Read the model definition and answer for the solid it produces. Units are mm, in the model's axes. Coordinates: 2 decimals unless noted, no trailing zeros. Order: outer loops, then holes, each group sorted by start corner. A loop starts at its lowest first (then second) coordinate and runs counter-clockwise, first axis right, second up. Notation, with made-up numbers: (28.25, 54.5) -> (33.25, 54.5) arc R15 cw to (33.25, 74.5) -> close; hole circle Ø3 at (47.25, 21). An arc over 180 degrees is marked (long way). Answer in a Markdown table with one row per item.
from build123d import *

# Parameters (mm, degrees)
SKETCH1_W           = 300
SKETCH1_H           = 80
BOSS_EXTRUDE1_DEPTH = 8
SKETCH2_R           = 4
CUT_EXTRUDE1_DEPTH  = 8
CHAMFER1_SIZE       = 5


with BuildPart() as part:
    # Sketch1 → Boss-Extrude1 (new body)
    with BuildSketch(Plane.XY):
        Rectangle(SKETCH1_W, SKETCH1_H)
    extrude(amount=BOSS_EXTRUDE1_DEPTH)

    # Sketch2 → Cut-Extrude1 (cut)
    with BuildSketch(Plane.XY.offset(8)):
        with Locations((-137.5, 25)):
            Circle(SKETCH2_R)
        with Locations((-137.5, -25)):
            Circle(SKETCH2_R)
        with Locations((137.5, 25)):
            Circle(SKETCH2_R)
        with Locations((137.5, -25)):
            Circle(SKETCH2_R)
    extrude(amount=-CUT_EXTRUDE1_DEPTH, mode=Mode.SUBTRACT)

    # Chamfer1
    chamfer1_edges = [part.edges().sort_by_distance(p)[0] for p in [
        (-150, -40, 4),
        (-150, 40, 4),
        (150, 40, 4),
        (150, -40, 4),
    ]]
    chamfer(chamfer1_edges, length=CHAMFER1_SIZE)


solid = part.part
Q1. For a pull along X with two mould halves and no side action, classify faces 1 (the face through (-147, 38, 4)), 2 (the face through (-133.685, -23.799, 4.056)), 3 (the face through (-2, -40, 4)) as pulls with the +X half, pulls with the -X half, needs draft (parallel to the pull), parting line crosses it, or undercut.
Outcome:
| item | result |
|---|---|
| face 1 | pulls with the -X half |
| face 2 | undercut |
| face 3 | needs draft |
Q2. The part is cut by section A-A (x = 137.5). Write down the section's boundary in (y, z), then the cut area to 3 significant figures.
Outcome:
| item | result |
|---|---|
| outline | (-40, 0) -> (-29, 0) -> (-29, 8) -> (-40, 8) -> close; (-21, 0) -> (21, 0) -> (21, 8) -> (-21, 8) -> close; (29, 0) -> (40, 0) -> (40, 8) -> (29, 8) -> close |
| area | 512 mm² |
Q3. Given pin 1 (6.5 mm diameter, centred on x = -137.5, y = -25, fed in from -Z), flat-ended and moving along its own axis, determine where the tip first touches the part or whether it passes through.
Outcome:
| item | result |
|---|---|
| pin 1 | through |
Q4. The part is cut by section B-B (y = 25). Write down the section's boundary in (x, z).
Outcome:
| item | result |
|---|---|
| outline | (-150, 0) -> (-141.5, 0) -> (-141.5, 8) -> (-150, 8) -> close; (-133.5, 0) -> (133.5, 0) -> (133.5, 8) -> (-133.5, 8) -> close; (141.5, 0) -> (150, 0) -> (150, 8) -> (141.5, 8) -> close |
Q5. Consider line 1 (Y direction, x = 137.5, z = 2.75); line 2 (X direction, y = 25.5, z = 4.5); line 3 (X direction, y = 28.5, z = 2.75). Determine where each line is inside the solid, lowest interval first.
Outcome:
| item | result |
|---|---|
| line 1 | -40 to -29, -21 to 21, 29 to 40 |
| line 2 | -150 to -141.47, -133.53 to 133.53, 141.47 to 150 |
| line 3 | -150 to -139.44, -135.56 to 135.56, 139.44 to 150 |
